Part model, mm, in its own coordinate system. A direction names the side the tool comes from. Coordinates: 2 decimals unless noted, no trailing zeros. Loops run counter-clockwise (first coordinate to the right, second up) from the corner with the lowest first, then second, coordinate; pieces in that order, holes last. Notation, with made-up numbers: M 36,2.5 L 75,2.5 A18 cw 75,25.5 Z; hole C -14,-35.5 d11. An arc over 180 degrees is marked long. Answer as a JSON object with one key per item and string values. Group by question number.
1. Saw through at D-D on z = 7. Write the cut outline in (x, y).
2. Saw through at C-C on z = 14. Write the cut outline in (x, y), then the cut area to 3 significant figures.
3. Mould opens along Y. For faces 1 (the face through (-0.2, -44.2, 0)), 2 (the face through (47.69, 15.02, 9.37)), 3 (the face through (-9.538, -42.954, 6.084)) say: released by +Y, released by -Y, zero draft, split by the parting line, or undercut.
4. Drop flat-ended pins along their axis: pin 1 Ø2 at (x, z) = (-21, 2.5) entering from -Y; pin 2 Ø4 at (y, z) = (-31, 5) entering from -X; pin 3 Ø4 at (y, z) = (-10.5, 10) entering from -X. Give the stop position or say it passes through.
5. Saw through at A-A on y = 0. Write the cut outline in (x, z).
6. 3-axis set-ups, long thin cutter, end or side, ignore diameter. For faces 4 (the face through (20.765, -39.923, 16.056)), 5 (the face through (22, -40, 20)): which of +Z, -Z, +X, -X, +Y, -Y reach the whole face in a straight line?
7. Drill centre lines: L1, parallel to Y at x = 0, z = 16; L2, parallel to X at y = -28, z = 11.5; L3, parallel to X at y = -30.5, z = 9.5. Where is each one in solid material? Low to high.
from build123d import *

# Parameters (mm, degrees)
RIM_OD_SKETCH_100_R       = 50
RIM_BLANK_100X20_DEPTH    = 20
RECESS_SKETCH_90_R        = 45
RECESS_90X8_DEPTH         = 8
BORE_SKETCH_88_R          = 44
BORE_88_THROUGH_DEPTH     = 50
EDGE_CHAMFER_1X45DEG_SIZE = 1


with BuildPart() as part:
    # Rim OD Sketch Ø100 → Rim Blank Ø100x20 (new body)
    with BuildSketch(Plane.XY):
        Circle(RIM_OD_SKETCH_100_R)
    extrude(amount=RIM_BLANK_100X20_DEPTH)

    # Recess Sketch Ø90 → Recess Ø90x8 (cut)
    with BuildSketch(Plane.XY.offset(20)):
        Circle(RECESS_SKETCH_90_R)
    extrude(amount=-RECESS_90X8_DEPTH, mode=Mode.SUBTRACT)

    # Bore Sketch Ø88 → Bore Ø88 Through (cut)
    with BuildSketch(Plane.XY.offset(12)):
        Circle(BORE_SKETCH_88_R)
    extrude(amount=-BORE_88_THROUGH_DEPTH, mode=Mode.SUBTRACT)

    # Edge Chamfer 1x45deg
    edge_chamfer_1x45deg_edges = [part.edges().sort_by_distance(p)[0] for p in [
        (-50, 0, 20),
    ]]
    chamfer(edge_chamfer_1x45deg_edges, length=EDGE_CHAMFER_1X45DEG_SIZE)


solid = part.part
Outcome:
{
 "1": {"outline": "C 0,0 d100; hole C 0,0 d88"},
 "2": {"outline": "C 0,0 d100; hole C 0,0 d90", "area": "1,490 mm²"},
 "3": {"face 1": "zero draft", "face 2": "split by the parting line", "face 3": "undercut"},
 "4": {"pin 1": "stops at y = -45.83", "pin 2": "stops at x = -40.73", "pin 3": "stops at x = -49.27"},
 "5": {"outline": "M -50,0 L -44,0 L -44,12 L -45,12 L -45,20 L -49,20 L -50,19 Z; M 44,0 L 50,0 L 50,19 L 49,20 L 45,20 L 45,12 L 44,12 Z"},
 "6": {"face 4": "+Z", "face 5": "+Z, +X, -X, +Y, -Y"},
 "7": {"L1": "y = -50 to -45, 45 to 50", "L2": "x = -41.42 to -33.94, 33.94 to 41.42", "L3": "x = -39.62 to -31.71, 31.71 to 39.62"}
}
